from build123d import *

# Parameters (mm, degrees)
SKETCH1_W                                            = 335
SKETCH1_H                                            = 15
BOSS_EXTRUDE1_DEPTH                                  = 10
CUT_EXTRUDE2_DEPTH                                   = 169.467355888
CBORE_FOR_M4_HEXAGON_SOCKET_HEAD_CAP_SCR_D           = 4.5
CBORE_FOR_M4_HEXAGON_SOCKET_HEAD_CAP_SCR_CBORE_D     = 8
CBORE_FOR_M4_HEXAGON_SOCKET_HEAD_CAP_SCR_CBORE_DEPTH = 4.6


with BuildPart() as part:
    # Sketch1 → Boss-Extrude1 (new body)
    with BuildSketch(Plane(origin=(0, 0, 0), x_dir=(0, 0, -1), z_dir=(1, 0, 0))):
        Rectangle(SKETCH1_W, SKETCH1_H)
    extrude(amount=BOSS_EXTRUDE1_DEPTH)

    # Sketch2 → Cut-Extrude2 (cut, through all)
    with BuildSketch(Plane.XZ.offset(7.5)):
        Polygon((8, 162.5), (8, -162.5), (10, -164), (10, 0), (10, 164), align=None)
    extrude(amount=-CUT_EXTRUDE2_DEPTH, mode=Mode.SUBTRACT)

    # CBORE for M4 Hexagon socket head cap screws1 (through all)
    with Locations(Plane(origin=(8, 0, 0), x_dir=(0, 0, -1), z_dir=(1, 0, 0))):
        with Locations((0, 0), (70, 0), (25, 0)):
            CounterBoreHole(CBORE_FOR_M4_HEXAGON_SOCKET_HEAD_CAP_SCR_D / 2, CBORE_FOR_M4_HEXAGON_SOCKET_HEAD_CAP_SCR_CBORE_D / 2, CBORE_FOR_M4_HEXAGON_SOCKET_HEAD_CAP_SCR_CBORE_DEPTH)


solid = part.part
Can you work these out from the model? Positions are in its coordinate system, mm. A direction names the side the tool comes from. Give positions to 0.01 mm unless a question says otherwise; leave off trailing zeros. Loops run counter-clockwise (first coordinate to the right, second up) from the corner with the lowest first, then second, coordinate; pieces in that order, holes last. Notation, with made-up numbers: (-15, -15.75) - (44, -15.75) arc R22 cw to (44, 17.25) - close; hole circle Ø11 at (-3, 88). An arc over 180 degrees is marked (long way). Return JSON: item names as keys, results as strings.
1. For faces 4 (the face through (3.4, -2, -27)), 5 (the face through (0, 2, 2)), 6 (the face through (8, -5, 2)), which set-ups out of +Z, -Z, +X, -X, +Y, -Y let a thin tool reach every point of the face, with its end or its side?
Output values:
{"face 4": "+X", "face 5": "+Z, -Z, -X, +Y, -Y", "face 6": "+X, +Y, -Y"}
2. If I drill on line 1 (Z direction, x = 6.75, y = 0.25); line 2 (Z direction, x = 6.5, y = 2); line 3 (Y direction, x = 5.1, z = 0), over which ranges is the centre line in solid material (lowest first)?
Output values:
{"line 1": "z = -167.5 to -73.99, -66.01 to -28.99, -21.01 to -3.99, 3.99 to 167.5", "line 2": "z = -167.5 to -73.46, -66.54 to -28.46, -21.54 to -3.46, 3.46 to 167.5", "line 3": "y = -7.5 to -4, 4 to 7.5"}
3. I want a section at B-B on y = 0. Give the number of separate pieces and of enclosed holes in the cut face, and give its area (3 significant figures).
Output values:
{"separate pieces": "4", "enclosed holes": "0", "area": "2,540 mm²"}
4. I want a section at A-A on x = 6.25. Please give me the cut outline in (y, z).
Output values:
{"outline": "(-7.5, -167.5) - (7.5, -167.5) - (7.5, 167.5) - (-7.5, 167.5) - close; hole circle Ø8 at (0, -70); hole circle Ø8 at (0, -25); hole circle Ø8 at (0, 0)"}
5. We'd pull the mould along Z, two halves only. Please class faces 1 (the face through (5, 0, 167.5)), 2 (the face through (5.732, -1.532, -73.695)), 3 (the face through (4, -7.5, 2)): +Z half, -Z half, draft (parallel to the pull), parting line (faces both ways), or undercut.
Output values:
{"face 1": "+Z half", "face 2": "undercut", "face 3": "draft"}
6. I want a section at C-C on z = 81.5. Please give me the cut outline in (x, y), and give its area (3 significant figures).
Output values:
{"outline": "(0, -7.5) - (8, -7.5) - (8, 7.5) - (0, 7.5) - close", "area": "120 mm²"}
7. I'm going to push flat-ended pins straight in: pin 1 Ø9 at (y, z) = (1, -26) entering from +X; pin 2 Ø4 at (y, z) = (0, 0) entering from +X; pin 3 Ø4 at (y, z) = (-1, 1) entering from +X. Where does each tip first touch, or does it pass through?
Output values:
{"pin 1": "stops at x = 8", "pin 2": "passes through", "pin 3": "stops at x = 3.4"}
